from build123d import *

# Parameters (mm, degrees)
SKETCH_1_W          = 30
SKETCH_1_H          = 30
SKETCH_1_W_2        = 26
SKETCH_1_H_2        = 26
EXTRUDE_1_DEPTH     = 150
CUT_EXTRUDE_1_DEPTH = 102


with BuildPart() as part:
    # 草图1 → 凸台-拉伸1 (new, symmetric)
    with BuildSketch(Plane.XY):
        Rectangle(SKETCH_1_W, SKETCH_1_H)
        Rectangle(SKETCH_1_W_2, SKETCH_1_H_2, mode=Mode.SUBTRACT)
    extrude(amount=EXTRUDE_1_DEPTH, both=True)

    # 草图3 → 切除-拉伸1 (cut)
    with BuildSketch(Plane(origin=(0, 15, 0), x_dir=(1, 0, 0), z_dir=(0, 1, 0))):
        Polygon((-15, 150), (0, 135), (15, 150), align=None)
    extrude(amount=-CUT_EXTRUDE_1_DEPTH, mode=Mode.SUBTRACT)


solid = part.part
Input: part model. Units: mm. Frame: model coordinates. A direction names the side the tool comes from. Coordinates: 2 decimals unless noted, no trailing zeros. Loops run counter-clockwise (first coordinate to the right, second up) from the corner with the lowest first, then second, coordinate; pieces in that order, holes last. Notation, with made-up numbers: (51, -6.75) -> (104, -6.75) arc R16 ccw to (104, 8.25) -> close; hole circle Ø7 at (51, -0.5). An arc over 180 degrees is marked (long way). Write each question's results on one line, items separated by ' | '. Start each with the question number.
Q1. Reachability of faces 5 (the flat face through (14, -1, -149)), 6 (the flat face through (0, 13, 3)), 7 (the flat face through (-14, 0, 150)) from +Z, -Z, +X, -X, +Y, -Y: full face, straight path, thin tool, end or side. Return the list, or none.
Q2. Ray query, line 1 (X direction, y = 8.5, z = -99); line 2 (Z direction, x = -14, y = -7). Return the intervals inside material, ascending. Write a range as from..to.
Q3. Section A-A, the plane y = -7. Return the cut outline in (x, z), plus the area to 3 significant figures.
Q4. Pull-direction query (Y, two-part tool) for faces 1 (the flat face through (0, -13, 3)), 2 (the flat face through (0, 15, 2)), 3 (the flat face through (0, -15, 2)), 4 (the flat face through (-14, 0, -149)); classes: released by +Y, released by -Y, zero draft, split by the parting line, or undercut.
Q5. Section C-C, the plane z = 69. Return the cut outline in (x, y), plus the area to 3 significant figures.
Q6. Section B-B, the plane x = 4.5. Return the cut outline in (y, z), plus the area to 3 significant figures.
Found:
1) face 5: -Z, +Y, -Y | face 6: +Z, -Z | face 7: +Z, +X, -X, +Y, -Y
2) line 1: -15..-13, 13..15 | line 2: -149..150
3) outline: (-15, -150) -> (-13, -148) -> (-13, 150) -> (-15, 150) -> close; (13, -148) -> (15, -150) -> (15, 150) -> (13, 150) -> close | area: 1,200 mm2
4) face 1: undercut | face 2: released by +Y | face 3: released by -Y | face 4: zero draft
5) outline: (-15, -15) -> (15, -15) -> (15, 15) -> (-15, 15) -> close; hole (-13, -13) -> (13, -13) -> (13, 13) -> (-13, 13) -> close | area: 224 mm2
6) outline: (-15, -139.5) -> (-13, -139.5) -> (-13, 150) -> (-15, 150) -> close; (13, -139.5) -> (15, -139.5) -> (15, 150) -> (13, 150) -> close | area: 1,160 mm2
